from build123d import *

# Parameters (mm, degrees)
SKETCH_1_W          = 333
SKETCH_1_H          = 436
EXTRUDE_1_DEPTH     = 3
SKETCH_3_W          = 30
SKETCH_3_H          = 90
CUT_EXTRUDE_2_DEPTH = 10
CUT_EXTRUDE_3_DEPTH = 10


with BuildPart() as part:
    # 草图1 → 凸台-拉伸1 (new body)
    with BuildSketch(Plane.XY):
        Rectangle(SKETCH_1_W, SKETCH_1_H)
    extrude(amount=EXTRUDE_1_DEPTH)

    # 草图3 → 切除-拉伸2 (cut)
    with BuildSketch(Plane(origin=(0, 0, 0), x_dir=(-1, 0, 0), z_dir=(0, 0, -1))):
        with Locations((-151.5, 173)):
            Rectangle(SKETCH_3_W, SKETCH_3_H)
    extrude(amount=-CUT_EXTRUDE_2_DEPTH, mode=Mode.SUBTRACT)

    # 草图4 → 切除-拉伸3 (cut)
    with BuildSketch(Plane.XY.offset(3)):
        with BuildLine():
            Line((-120, 201.7), (-126, 201.7))
            ThreePointArc((-126, 201.7), (-129.3, 205), (-126, 208.3))
            Line((-126, 208.3), (-120, 208.3))
            ThreePointArc((-120, 208.3), (-116.7, 205), (-120, 201.7))
        make_face()
        with BuildLine():
            Line((120, 208.3), (126, 208.3))
            ThreePointArc((126, 208.3), (129.3, 205), (126, 201.7))
            Line((126, 201.7), (120, 201.7))
            ThreePointArc((120, 201.7), (116.7, 205), (120, 208.3))
        make_face()
        with BuildLine():
            Line((120, -201.7), (126, -201.7))
            ThreePointArc((126, -201.7), (129.3, -205), (126, -208.3))
            Line((126, -208.3), (120, -208.3))
            ThreePointArc((120, -208.3), (116.7, -205), (120, -201.7))
        make_face()
        with BuildLine():
            Line((-120, -208.3), (-126, -208.3))
            ThreePointArc((-126, -208.3), (-129.3, -205), (-126, -201.7))
            Line((-126, -201.7), (-120, -201.7))
            ThreePointArc((-120, -201.7), (-116.7, -205), (-120, -208.3))
        make_face()
    extrude(amount=-CUT_EXTRUDE_3_DEPTH, mode=Mode.SUBTRACT)


solid = part.part
The listing builds one solid part. Answer for the finished solid, in the listing's coordinates (mm). Coordinates: 2 decimals unless noted, no trailing zeros. Order: outer loops, then holes, each group sorted by start corner. A loop starts at its lowest first (then second) coordinate and runs counter-clockwise, first axis right, second up.
Q1. Given P1, Ø1.5, axis at x = 148.5, z = 2, coming from the +Y side; P2, Ø1.5, axis at y = 185.5, z = 1, coming from the +X side, each flat-ended and moving along its own axis, determine where each tip first touches the part or whether it passes through.
Q2. A cutting plane is placed at B-B, the plane x = 144.5. Write down the section's boundary in (y, z), and give its area (3 significant figures).
Q3. Consider line 1 (X direction, y = 144.5, z = 2.85). Determine where the line is inside the solid, lowest interval first.
Q4. A cutting plane is placed at A-A, the plane z = 0.7. Write down the section's boundary in (x, y), and give its area (3 significant figures).
Q5. A cutting plane is placed at C-C, the plane y = 134. Write down the section's boundary in (x, z), and give its area (3 significant figures).
Answers follow:
1. P1: stops at y = 128
1. P2: stops at x = 136.5
2. outline: (-218, 0) - (128, 0) - (128, 3) - (-218, 3) - close
2. area: 1,040 mm2
3. line 1: x = -166.5 to 136.5
4. outline: (-166.5, -218) - (166.5, -218) - (166.5, 128) - (136.5, 128) - (136.5, 218) - (-166.5, 218) - close; hole (-126, -208.3) - (-120, -208.3) arc R3.3 ccw to (-120, -201.7) - (-126, -201.7) arc R3.3 ccw to start; hole (-126, 201.7) - (-120, 201.7) arc R3.3 ccw to (-120, 208.3) - (-126, 208.3) arc R3.3 ccw to start; hole (120, -208.3) - (126, -208.3) arc R3.3 ccw to (126, -201.7) - (120, -201.7) arc R3.3 ccw to start; hole (120, 201.7) - (126, 201.7) arc R3.3 ccw to (126, 208.3) - (120, 208.3) arc R3.3 ccw to start
4. area: 142,000 mm2
5. outline: (-166.5, 0) - (136.5, 0) - (136.5, 3) - (-166.5, 3) - close
5. area: 909 mm2
